The model under review builds one solid part; all positions refer to its coordinate system, in mm. Face numbers are marked on the shaded views. A direction names the side the tool comes from. Coordinates: 2 decimals unless noted, no trailing zeros. Order: outer loops, then holes, each group sorted by start corner. A loop starts at its lowest first (then second) coordinate and runs counter-clockwise, first axis right, second up. Notation, with made-up numbers: (12, 30.25) - (18, 30.25) arc R23 cw to (18, 67.25) - close; hole circle Ø6 at (-30, -28). An arc over 180 degrees is marked (long way). Answer in a Markdown table with one row per item.
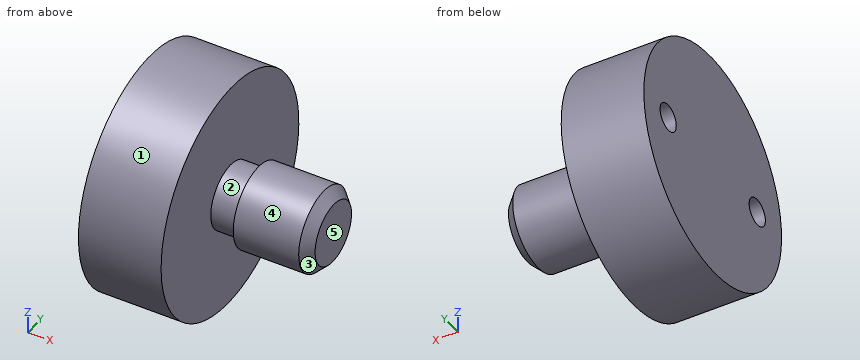
```python
from build123d import *

# Parameters (mm, degrees)
CHAMFER1_SIZE = 1.5


with BuildPart() as part:
    # Sketch1 → Revolve1 (revolve)
    with BuildSketch(Plane.XY, mode=Mode.PRIVATE) as revolve1_sk:
        Polygon((0, 0), (0, 17), (12, 17), (12, 4.75), (16, 4.75), (16, 6), (27, 6), (27, 0), align=None)
    revolve(revolve1_sk.sketch.rotate(Axis((0, 0, 0), (1, 0, 0)), 90), axis=Axis((0, 0, 0), (1, 0, 0)))

    # Chamfer1
    chamfer1_edges = [part.edges().sort_by_distance(p)[0] for p in [
        (27, 0, -6),
    ]]
    chamfer(chamfer1_edges, length=CHAMFER1_SIZE)

    # Sketch2 → Cut-Revolve1 (revolve, cut)
    with BuildSketch(Plane.XY, mode=Mode.PRIVATE) as cut_revolve1_sk:
        Polygon((0, 11), (0, 13), (6, 13), (7.154700538, 11), align=None)
    cut_revolve1 = revolve(cut_revolve1_sk.sketch.rotate(Axis((-2.466856423, 11, 0), (1, 0, 0)), 90), axis=Axis((-2.466856423, 11, 0), (1, 0, 0)), mode=Mode.SUBTRACT)

    # Mirror1: Cut-Revolve1 across plane
    add(cut_revolve1.mirror(Plane.ZX), mode=Mode.SUBTRACT)


solid = part.part
```
Item 1: Mouldability with a two-part tool opening along X and no side actions: class the marked faces 1, 2 and 3 as +X half, -X half, draft (parallel to the pull), parting line (faces both ways), or undercut.
Check values:
| item | result |
|---|---|
| face 1 | draft |
| face 2 | undercut |
| face 3 | +X half |
Item 2: We need section A-A, the plane y = 0. Write out the cut boundary in (x, z).
Check values:
| item | result |
|---|---|
| outline | (0, -17) - (12, -17) - (12, -4.75) - (16, -4.75) - (16, -6) - (25.5, -6) - (27, -4.5) - (27, 4.5) - (25.5, 6) - (16, 6) - (16, 4.75) - (12, 4.75) - (12, 17) - (0, 17) - close |
Item 3: We need section B-B, the plane x = 22. Write out the cut boundary in (y, z).
Check values:
| item | result |
|---|---|
| outline | circle Ø12 at (0, 0) |
Item 4: We need section C-C, the plane z = 10. Write out the cut boundary in (x, y).
Check values:
| item | result |
|---|---|
| outline | (0, -13.75) - (12, -13.75) - (12, 13.75) - (0, 13.75) - close |
Item 5: To check wall thickness, follow line 1 (Y direction, x = 3.3, z = 0); line 2 (X direction, y = -0.5, z = 9); line 3 (Z direction, x = 4.3, y = 11). State the ranges of each line that lie inside material, in increasing order. Write a range as from..to.
Check values:
| item | result |
|---|---|
| line 1 | -17..-13, -9..9, 13..17 |
| line 2 | 0..12 |
| line 3 | -12.96..-2, 2..12.96 |
Item 6: Clearance check with flat-ended pins moving along their axes: pin 1 Ø2.5 at (y, z) = (11, 0) entering from +X; pin 2 Ø12 at (x, z) = (7, 12.5) entering from +Y; pin 3 Ø1.5 at (x, y) = (14.5, -7) entering from -Z; pin 4 Ø3 at (x, y) = (8, 8) entering from +Z. State where each tip first meets the part, or that it passes through.
Check values:
| item | result |
|---|---|
| pin 1 | x = 12 |
| pin 2 | y = 15.71 |
| pin 3 | through |
| pin 4 | z = 15.71 |
Item 7: We need section D-D, the plane x = 14.75. Write out the cut boundary in (y, z), then the cut area to 3 significant figures.
Check values:
| item | result |
|---|---|
| outline | circle Ø9.5 at (0, 0) |
| area | 70.9 mm^2 |
Item 8: Tool access review of the marked faces 4 and 5: name each direction out of +Z, -Z, +X, -X, +Y, -Y from which nothing blocks a thin tool from reaching the whole face with its end or side.
Check values:
| item | result |
|---|---|
| face 4 | +X |
| face 5 | +Z, -Z, +X, +Y, -Y |
